Print and shaded views of the part. All mm, measured from the part's lowest x, y and z. Round coordinates to 2 decimals unless told otherwise and drop trailing zeros. Loops run counter-clockwise (first coordinate to the right, second up) from the corner with the lowest first, then second, coordinate; pieces in that order, holes last. Notation, with made-up numbers: (37.5, 49.5) - (53.5, 49.5) arc R19 cw to (53.5, 66.5) - close; hole circle Ø5 at (10.25, -7.75). An arc over 180 degrees is marked (long way). Use one line per item in the form item = value. Start each with the question number.
Q1. Mould opens along X. For the marked faces 1 and 2 say: released by +X, released by -X, zero draft, split by the parting line, or undercut.
Q2. Saw through at B-B (x = 50). Give the cut face in (y, z).
Q3. Saw through at A-A (z = 50). Give the cut face in (x, y).
Q4. Saw through at C-C (y = 5.25). Give the cut face in (x, z).
Q5. Drill centre lines: line 1 (X direction, y = 4.5, z = 50); line 2 (Z direction, x = 50, y = 4.5); line 3 (X direction, y = 1, z = 47.5). Where is each one in solid material? Low to high.
Q6. Pin check, flat tip, straight feed: pin 1 (1.5 mm diameter, centred on y = 6.5, z = 16, fed in from +X). Stop position of the tip, or through.
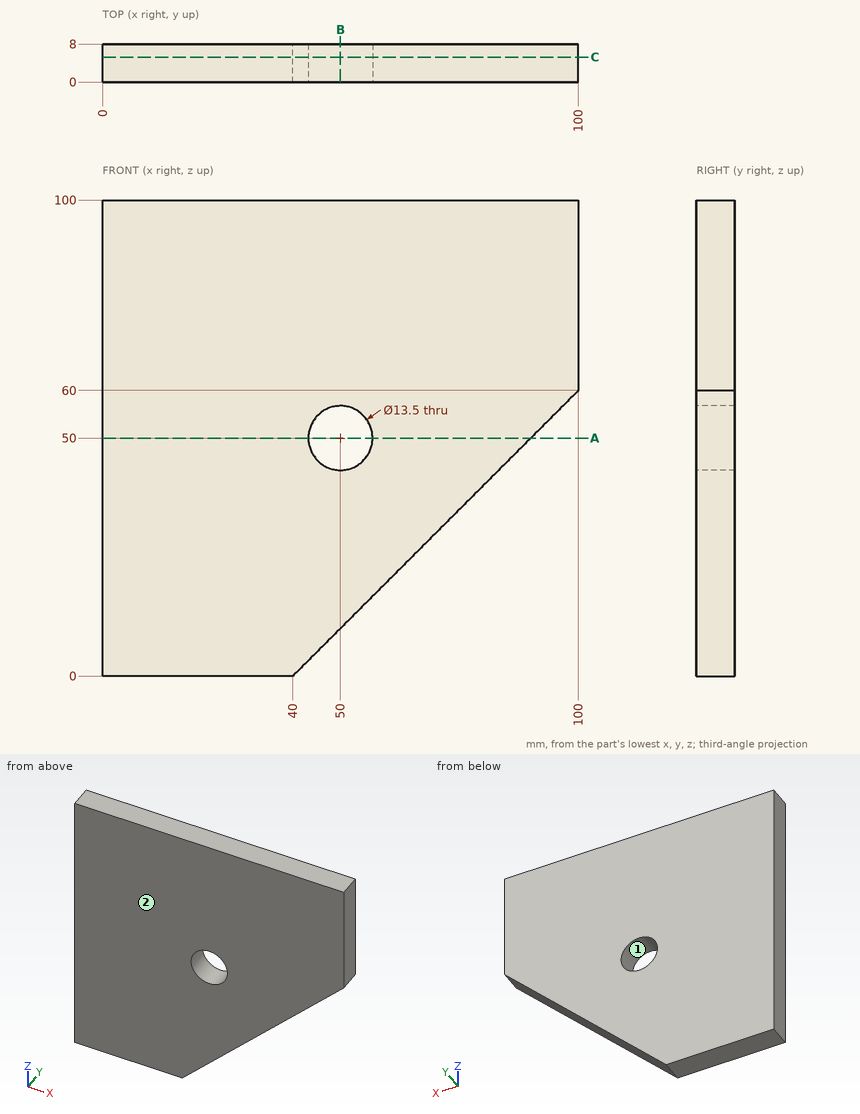
Report:
q1.face_1 = undercut
q1.face_2 = zero draft
q2.outline = (0, 10) - (8, 10) - (8, 43.25) - (0, 43.25) - close; (0, 56.75) - (8, 56.75) - (8, 100) - (0, 100) - close
q3.outline = (0, 0) - (43.25, 0) - (43.25, 8) - (0, 8) - close; (56.75, 0) - (90, 0) - (90, 8) - (56.75, 8) - close
q4.outline = (0, 0) - (40, 0) - (100, 60) - (100, 100) - (0, 100) - close; hole circle Ø13.5 at (50, 50)
q5.line_1 = 0 to 43.25, 56.75 to 90
q5.line_2 = 10 to 43.25, 56.75 to 100
q5.line_3 = 0 to 43.73, 56.27 to 87.5
q6.pin_1 = 56.75
